Input: part model. Units: mm. Frame: model coordinates. Coordinates: 2 decimals unless noted, no trailing zeros. Loops run counter-clockwise (first coordinate to the right, second up) from the corner with the lowest first, then second, coordinate; pieces in that order, holes last.
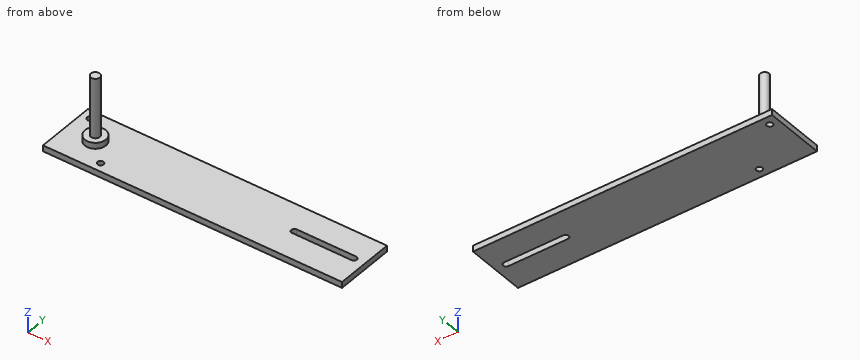
```python
from build123d import *

# Parameters (mm, degrees)
SKETCH1_W           = 500
SKETCH1_H           = 100
BOSS_EXTRUDE1_DEPTH = 10
CUT_EXTRUDE1_DEPTH  = 60
SKETCH4_R           = 5
CUT_EXTRUDE2_DEPTH  = 60
SKETCH2_R           = 17.5
BOSS_EXTRUDE2_DEPTH = 60
CUT_EXTRUDE3_START  = -50
SKETCH5_R           = 17.5
SKETCH5_R_2         = 7.5
CUT_EXTRUDE3_DEPTH  = 50
SKETCH6_R           = 7.5
BOSS_EXTRUDE3_DEPTH = 50


with BuildPart() as part:
    # Sketch1 → Boss-Extrude1 (new body)
    with BuildSketch(Plane.XY):
        Rectangle(SKETCH1_W, SKETCH1_H)
    extrude(amount=BOSS_EXTRUDE1_DEPTH)

    # Sketch3 → Cut-Extrude1 (cut)
    with BuildSketch(Plane.XY.offset(10)):
        with BuildLine():
            Line((231.804981109, -3.932202525), (131.558181165, -3.932202525))
            ThreePointArc((131.558181165, -3.932202525), (128.376200649, -2.614183041), (127.058181165, 0.567797475))
            Line((127.058181165, 0.567797475), (127.058181165, 1.567797475))
            ThreePointArc((127.058181165, 1.567797475), (128.376200649, 4.74977799), (131.558181165, 6.067797475))
            Line((131.558181165, 6.067797475), (231.804981109, 6.067797475))
            ThreePointArc((231.804981109, 6.067797475), (234.986961624, 4.74977799), (236.304981109, 1.567797475))
            Line((236.304981109, 1.567797475), (236.304981109, 0.567797475))
            ThreePointArc((236.304981109, 0.567797475), (234.986961624, -2.614183041), (231.804981109, -3.932202525))
        make_face()
    extrude(amount=-CUT_EXTRUDE1_DEPTH, mode=Mode.SUBTRACT)

    # Sketch4 → Cut-Extrude2 (cut)
    with BuildSketch(Plane.XY.offset(10)):
        with Locations((-235, 35)):
            Circle(SKETCH4_R)
        with Locations((-165, -35)):
            Circle(SKETCH4_R)
    extrude(amount=-CUT_EXTRUDE2_DEPTH, mode=Mode.SUBTRACT)

    # Sketch2 → Boss-Extrude2 (add)
    with BuildSketch(Plane.XY.offset(10)):
        with Locations(Location((-200, 0, 0), (0, 0, 180))):
            Circle(SKETCH2_R)
    extrude(amount=BOSS_EXTRUDE2_DEPTH)

    # Sketch5 → Cut-Extrude3 (cut)
    with BuildSketch(Plane.XY.offset(70).offset(CUT_EXTRUDE3_START)):
        with Locations(Location((-200, 0, 0), (0, 0, 180))):
            Circle(SKETCH5_R)
        with Locations((-200, 0)):
            Circle(SKETCH5_R_2, mode=Mode.SUBTRACT)
    extrude(amount=CUT_EXTRUDE3_DEPTH, mode=Mode.SUBTRACT)

    # Sketch6 → Boss-Extrude3 (add)
    with BuildSketch(Plane.XY.offset(70)):
        with Locations((-200, 0)):
            Circle(SKETCH6_R)
    extrude(amount=BOSS_EXTRUDE3_DEPTH)


solid = part.part
```
Item 1: Section query B-B (x = -235). Output: boundary loops of the cut face in (y, z).
Result:
outline: (-50, 0) - (30, 0) - (30, 10) - (-50, 10) - close; (40, 0) - (50, 0) - (50, 10) - (40, 10) - close
Item 2: Section query A-A (y = 35). Output: boundary loops of the cut face in (x, z), then the cut area to 3 significant figures.
Result:
outline: (-250, 0) - (-240, 0) - (-240, 10) - (-250, 10) - close; (-230, 0) - (250, 0) - (250, 10) - (-230, 10) - close
area: 4,900 mm2
Item 3: Contact query for flat-ended pins moving along their axis: P1, Ø1.5, axis at x = 42, z = 12.5, coming from the -Y side; P2, Ø16, axis at x = -165, y = -35, coming from the +Z side; P3, Ø4, axis at y = 7.5, z = 39, coming from the +X side; P4, Ø5, axis at y = -1, z = 61, coming from the +X side. Output: stop coordinate, or through.
Result:
P1: passes through
P2: stops at z = 10
P3: stops at x = -194.9
P4: stops at x = -192.5
Item 4: Section query C-C (z = 36). Output: boundary loops of the cut face in (x, y), then the cut area to 3 significant figures.
Result:
outline: circle Ø15 at (-200, 0)
area: 177 mm2
Item 5: Line query: L1, parallel to Y at x = -165, z = 3.5; L2, parallel to Y at x = -235, z = 2.25; L3, parallel to Z at x = 152.5, y = 21. Output: solid intervals per line, ascending.
Result:
L1: y = -50 to -40, -30 to 50
L2: y = -50 to 30, 40 to 50
L3: z = 0 to 10
Item 6: Section query D-D (x = -105). Output: boundary loops of the cut face in (y, z).
Result:
outline: (-50, 0) - (50, 0) - (50, 10) - (-50, 10) - close
